Source: CAD feature listing. Evaluate the final solid. Frame: model axes, mm. A direction names the side the tool comes from. Give positions to 0.01 mm unless a question says otherwise; leave off trailing zeros. Order: outer loops, then holes, each group sorted by start corner. A loop starts at its lowest first (then second) coordinate and runs counter-clockwise, first axis right, second up. Notation, with made-up numbers: (23, 14) -> (70, 14) arc R21 ccw to (70, 51) -> close; hole circle Ø8 at (48, -31.5). An arc over 180 degrees is marked (long way). Use CSV: the item, a comma, the result in double quotes.
```python
from build123d import *

# Parameters (mm, degrees)
TROUGH_SHELL_DEPTH      = 20
TROUGH_SHELL_DEPTH_BACK = 5
END_START               = -5
END_PLATE_DEPTH         = 5
SIDE_WALLS_REACH        = 316.327


with BuildPart() as part:
    # Trough Profile Sketch → Trough Shell (new, two sides: drawn at the far end of the back side and taken through both)
    with BuildSketch(Plane.XY.offset(-TROUGH_SHELL_DEPTH_BACK)):
        with BuildLine():
            Line((0, 17), (0, 25))
            ThreePointArc((0, 25), (-25, 0), (0, -25))
            Line((0, -25), (0, -17))
            ThreePointArc((0, -17), (-17, 0), (0, 17))
        make_face()
    extrude(amount=TROUGH_SHELL_DEPTH + TROUGH_SHELL_DEPTH_BACK)

    # End Plate Sketch → End Plate (add)
    with BuildSketch(Plane.XY.offset(END_START)):
        with BuildLine():
            Line((0, 25), (0, 77))
            Line((0, 77), (-65, 77))
            Line((-65, 77), (-65, 32.113081447))
            ThreePointArc((-65, 32.113081447), (-61.581037686, -38.262590053), (0, -72.5))
            Line((0, -72.5), (0, -25))
            ThreePointArc((0, -25), (-25, 0), (0, 25))
        make_face()
    extrude(amount=END_PLATE_DEPTH)


with BuildPart() as body_2:
    # End Plate Mirror: mirrored copy
    add(part.part.mirror(Plane.XY.offset(-140.5)))

    # Side Wall Sketch → Side Walls (add, up to next)
    with BuildSketch(Plane(origin=(0, 0, -5), x_dir=(-1, 0, 0), z_dir=(0, 0, -1)), mode=Mode.PRIVATE) as side_walls_sk1:
        with BuildLine():
            Line((65, 77), (65, 32.113081447))
            ThreePointArc((65, 32.113081447), (61.581037686, -38.262590053), (0, -72.5))
            Line((0, -72.5), (0, -67.5))
            ThreePointArc((0, -67.5), (57.634938288, -35.134938288), (60, 30.923292192))
            Line((60, 30.923292192), (60, 77))
            Line((60, 77), (65, 77))
        make_face()
    side_walls_tool1 = extrude(side_walls_sk1.sketch, amount=SIDE_WALLS_REACH, mode=Mode.PRIVATE) - body_2.part

    add(part.part)  # Side Walls merges part
    add(side_walls_tool1.solids().sort_by_distance((-61.66152, 53.961646, -5))[0])


solid = body_2.part
```
1. Ray query, line 1 along Z through (x, y) = (-18.5, -18.5); line 2 along X through (y, z) = (58, -124); line 3 along Z through (x, y) = (-69, -3.5). Return the intervals inside material, ascending.
Answer below:
line 1,"z = -281 to -276, -5 to 0"
line 2,"x = -65 to -60"
line 3,"z = -281 to 0"
2. Access query for faces 4 (the cylindrical face through (-24.994, 0.55, -290.86)), 5 (the cylindrical face through (-17, 0, 7)), 6 (the cylindrical face through (-57.1, -36, -138.6)), 7 (the flat face through (-37, 3, 0)), 8 (the flat face through (-60, 54, -139)). Directions: +Z, -Z, +X, -X, +Y, -Y. A direction counts if a zero-diameter tool reaches every point of the face in a straight line with its end or side. Return the directions, or none.
Answer below:
face 4,"-Z, -X"
face 5,"+Z, -Z, +X"
face 6,"+X"
face 7,"+Z, -X"
face 8,"+X, +Y"
3. Section query D-D on y = 52. Return loops of the section in (x, z).
Answer below:
outline,"(-65, -281) -> (0, -281) -> (0, -276) -> (-60, -276) -> (-60, -5) -> (0, -5) -> (0, 0) -> (-65, 0) -> close"
4. Pin query (flat end, axial travel): P1, Ø12, axis at y = -13, z = -220, coming from the +X side; P2, Ø5, axis at x = -48.5, z = -111, coming from the +Y side; P3, Ø8, axis at y = -52, z = -59.5, coming from the +X side. Return the tip coordinate at first contact, or that it passes through.
Answer below:
P1,"stops at x = -64.77"
P2,"stops at y = -44.22"
P3,"stops at x = -37.69"
5. Section query A-A on y = 0. Return loops of the section in (x, z), plus the area to 3 significant figures.
Answer below:
outline,"(-72.5, -281) -> (-25, -281) -> (-25, -301) -> (-17, -301) -> (-17, -276) -> (-67.5, -276) -> (-67.5, -5) -> (-17, -5) -> (-17, 20) -> (-25, 20) -> (-25, 0) -> (-72.5, 0) -> close"
area,"2,230 mm²"
6. Section query B-B on z = -216.5. Return loops of the section in (x, y).
Answer below:
outline,"(-65, 32.11) arc R72.5 ccw to (0, -72.5) -> (0, -67.5) arc R67.5 cw to (-60, 30.92) -> (-60, 77) -> (-65, 77) -> close"
7. Section query C-C on x = -29. Return loops of the section in (y, z), plus the area to 3 significant figures.
Answer below:
outline,"(-66.45, -281) -> (77, -281) -> (77, -276) -> (-60.95, -276) -> (-60.95, -5) -> (77, -5) -> (77, 0) -> (-66.45, 0) -> close"
area,"2,920 mm²"
8. Mould query, pull axis Y, two halves, no side actions, for faces 1 (the cylindrical face through (-17, 0, -288)), 2 (the cylindrical face through (-62.12, -37.38, -138.53)), 3 (the flat face through (-65, 55, -139)). Classes: released by +Y, released by -Y, zero draft, split by the parting line, or undercut.
Answer below:
face 1,"undercut"
face 2,"split by the parting line"
face 3,"zero draft"
